from build123d import *

# Parameters (mm, degrees)
BOSS_EXTRUDE1_DEPTH = 25


with BuildPart() as part:
    # Sketch1 → Boss-Extrude1 (new body)
    with BuildSketch(Plane.XY):
        Polygon((0, 0), (20, 0), (100, 80), (100, 100), (20, 100), (0, 80), align=None)
    extrude(amount=BOSS_EXTRUDE1_DEPTH)


solid = part.part
Source: CAD feature listing. Evaluate the final solid. Frame: model axes, mm. Give positions to 0.01 mm unless a question says otherwise; leave off trailing zeros. Write each loop counter-clockwise with the first axis right and the second up, starting at its lowest first coordinate (ties: lowest second). Pieces come first, ordered by that corner, then holes. Notation, with made-up numbers: (72.5, -15.75) - (81.5, -15.75) arc R11 ccw to (81.5, 3.25) - close; hole circle Ø8 at (76.25, -8.75). An arc over 180 degrees is marked (long way). Write item = value, one per line. Start each with the question number.
Q1. Pin query (flat end, axial travel): pin 1 Ø5 at (y, z) = (14.5, 11.5) entering from +X; pin 2 Ø2 at (x, y) = (61.5, 70.5) entering from -Z; pin 3 Ø8 at (x, z) = (41.5, 11) entering from -Y. Return the tip coordinate at first contact, or that it passes through.
Q2. Material intervals for probe 1 along X at (y, z) = (60, 7.5); probe 2 along Y at (x, z) = (86, 5.75); probe 3 along Y at (x, z) = (68, 1.75), sorted ascending.
Q3. Cut plane C-C, the plane x = 41. Return loops of the section in (y, z), then the cut area to 4 significant figures.
Q4. Cut plane A-A, the plane z = 21.25. Return loops of the section in (x, y).
Q5. Cut plane B-B, the plane y = 86. Return loops of the section in (x, z), then the cut area to 3 significant figures.
Computed values:
q1.pin_1 = 37
q1.pin_2 = 0
q1.pin_3 = 17.5
q2.probe_1 = 0 to 80
q2.probe_2 = 66 to 100
q2.probe_3 = 48 to 100
q3.outline = (21, 0) - (100, 0) - (100, 25) - (21, 25) - close
q3.area = 1,975 mm²
q4.outline = (0, 0) - (20, 0) - (100, 80) - (100, 100) - (20, 100) - (0, 80) - close
q5.outline = (6, 0) - (100, 0) - (100, 25) - (6, 25) - close
q5.area = 2,350 mm²
